Design review of the part shown in the three views and the two pictorial views. Dimensions are in mm from the part's minimum x, y and z. A direction names the side the tool comes from. Round coordinates to 2 decimals unless told otherwise and drop trailing zeros. Loops run counter-clockwise (first coordinate to the right, second up) from the corner with the lowest first, then second, coordinate; pieces in that order, holes last. Notation, with made-up numbers: M 48,22 L 57,22 A28 cw 57,56 Z; hole C 74,39.25 d4. An arc over 180 degrees is marked long. Return JSON: item names as keys, results as strings. Group by question number.
Q1. Clearance check with flat-ended pins moving along their axes: pin 1 Ø6 at (y, z) = (49.5, 3) entering from -X; pin 2 Ø10 at (x, z) = (13.5, 15.5) entering from +Y; pin 3 Ø2 at (x, y) = (75.5, 39.5) entering from +Z; pin 4 Ø1.5 at (y, z) = (6, 16) entering from +X. State where each tip first meets the part, or that it passes through.
Q2. Consider section A-A (z = 20.5). State the section outline as (x, y) points.
Q3. Consider section D-D (z = 7.25). State the section outline as (x, y) points, and give its area (3 significant figures).
Q4. To check wall thickness, follow line 1 along Y through (x, z) = (62, 3); line 2 along Z through (x, y) = (22, 26.5); line 3 along Y through (x, z) = (11, 20). State the ranges of each line that lie inside material, in increasing order.
Q5. For the marked faces 4, 5, 6, 7 and 8, list the 3-axis set-ups (+Z, -Z, +X, -X, +Y, -Y) from which the entire face can be reached by the end or side of a thin tool; tool diameter is ignored.
Q6. Consider section C-C (x = 47). State the section outline as (y, z) points, and give its area (3 significant figures).
Q7. Draft analysis for pull direction Y (two halves, no side actions). For the marked faces 1, 2 and 3, state which applies: pulls with the +Y half, pulls with the -Y half, needs draft (parallel to the pull), parting line crosses it, or undercut.
Q8. Consider section B-B (y = 45). State the section outline as (x, z) points.
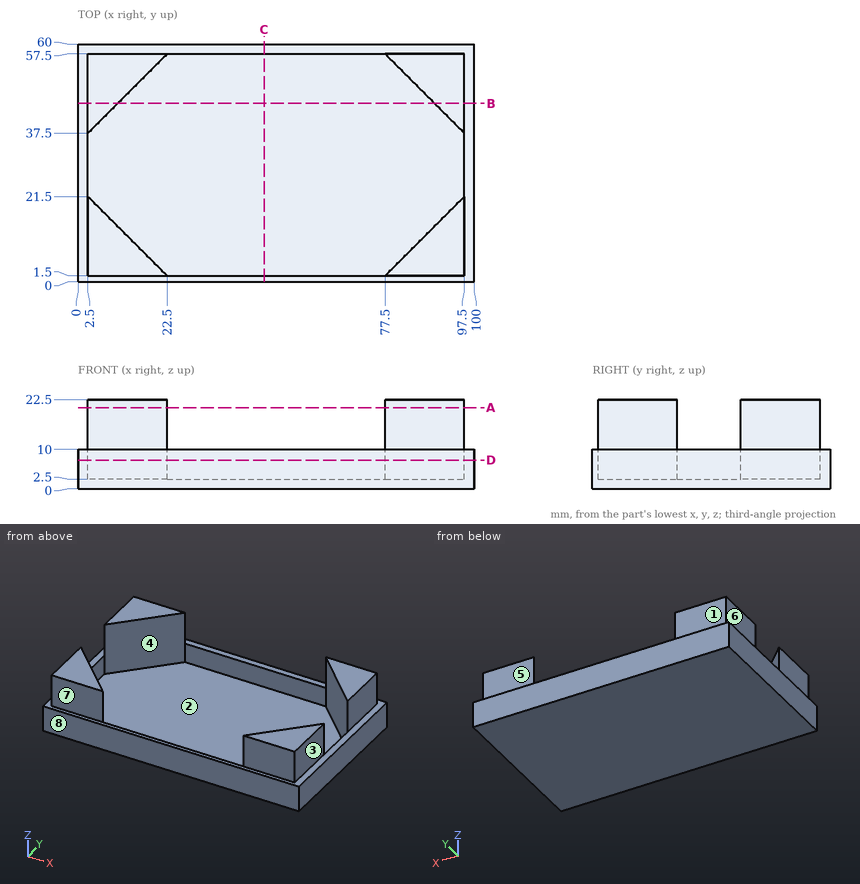
Values:
{
 "1": {"pin 1": "stops at x = 0", "pin 2": "stops at y = 57.5", "pin 3": "stops at z = 2.5", "pin 4": "stops at x = 97.5"},
 "2": {"outline": "M 2.5,1.5 L 22.5,1.5 L 2.5,21.5 Z; M 2.5,37.5 L 22.5,57.5 L 2.5,57.5 Z; M 77.5,1.5 L 97.5,1.5 L 97.5,21.5 Z; M 77.5,57.5 L 97.5,37.5 L 97.5,57.5 Z"},
 "3": {"outline": "M 0,0 L 100,0 L 100,60 L 0,60 Z; hole M 2.5,21.5 L 22.5,1.5 L 77.5,1.5 L 97.5,21.5 L 97.5,37.5 L 77.5,57.5 L 22.5,57.5 L 2.5,37.5 Z", "area": "1,480 mm2"},
 "4": {"line 1": "y = 0 to 1.5, 57.5 to 60", "line 2": "z = 0 to 2.5", "line 3": "y = 1.5 to 13, 46 to 57.5"},
 "5": {"face 4": "+Z", "face 5": "+Z, +X, -X, +Y", "face 6": "+Z, -X, +Y, -Y", "face 7": "+Z, +X, -X, -Y", "face 8": "+Z, -Z, +X, -X, -Y"},
 "6": {"outline": "M 0,0 L 60,0 L 60,10 L 57.5,10 L 57.5,2.5 L 1.5,2.5 L 1.5,10 L 0,10 Z", "area": "180 mm2"},
 "7": {"face 1": "pulls with the +Y half", "face 2": "undercut", "face 3": "needs draft"},
 "8": {"outline": "M 0,0 L 100,0 L 100,10 L 97.5,10 L 97.5,22.5 L 90,22.5 L 90,2.5 L 10,2.5 L 10,22.5 L 2.5,22.5 L 2.5,10 L 0,10 Z"}
}
